Geometry: final body of the model. Coordinates: model frame, mm. A direction names the side the tool comes from. Coordinates: 2 decimals unless noted, no trailing zeros. Order: outer loops, then holes, each group sorted by start corner. A loop starts at its lowest first (then second) coordinate and runs counter-clockwise, first axis right, second up. Notation, with made-up numbers: M -14,-30 L 26,-30 A16 ccw 26,-20 Z; hole C 55.5,41 d10. An arc over 180 degrees is marked long. Use CSV: the item, a comma, the result in double quotes. Start each with the question number.
1. Section query C-C on z = 1.7. Return the cut outline in (x, y), and give its area (3 significant figures).
2. Set-up query: faces 1 (the flat face through (0, 0, 3)), 2 (the flat face through (13, -2.75, 2)). Return all of +Z, -Z, +X, -X, +Y, -Y with unobstructed straight access to the full face (end or side cutting, diameter ignored); none if empty.
3. First-contact query: P1, Ø1, axis at y = 5.5, z = 2.5, coming from the +X side; P2, Ø4.5, axis at x = -17.5, y = 0, coming from the -Z side. Flat tips, straight axial feed; report the tip coordinate or a pass-through.
4. Pull-direction query (Y, two-part tool) for faces 3 (the flat face through (21, 6, 1)), 4 (the flat face through (-21, -6, 1)), 5 (the cylindrical face through (20.25, 0.06, 1.52)), 6 (the cylindrical face through (4.75, -0.06, 1.52)); classes: pulls with the +Y half, pulls with the -Y half, needs draft (parallel to the pull), parting line crosses it, or undercut.
5. Section query A-A on x = 13.5. Return the cut outline in (y, z), and give its area (3 significant figures).
6. Section query B-B on y = 0. Return the cut outline in (x, z).
7. Section query D-D on x = -17.5. Return the cut outline in (y, z), and give its area (3 significant figures).
8. Material intervals for line 1 (Y direction, x = -17.5, z = 1.1); line 2 (X direction, y = 0.5, z = 0.9); line 3 (Y direction, x = 20, z = 0.25), sorted ascending.
from build123d import *

# Parameters (mm, degrees)
SKETCH1_W             = 45
SKETCH1_H             = 15
BOSS_EXTRUDE1_DEPTH   = 3
M4_TAPPED_HOLE1_D     = 3.3
M4_TAPPED_HOLE1_DEPTH = 10.1
M4_TAPPED_HOLE1_TIP   = 0.991420021
CUT_EXTRUDE1_DEPTH    = 3
CHAMFER1_SIZE         = 3
CHAMFER2_SIZE         = 0.5


with BuildPart() as part:
    # Sketch1 → Boss-Extrude1 (new body)
    with BuildSketch(Plane.XY):
        Rectangle(SKETCH1_W, SKETCH1_H)
    extrude(amount=BOSS_EXTRUDE1_DEPTH)

    # M4 Tapped Hole1
    with Locations(Plane.XY.offset(3)):
        with Locations((-17.5, 0)):
            Hole(M4_TAPPED_HOLE1_D / 2, depth=M4_TAPPED_HOLE1_DEPTH)
            with Locations((0, 0, -(M4_TAPPED_HOLE1_DEPTH + M4_TAPPED_HOLE1_TIP / 2))):  # 118° drill point
                Cone(0, M4_TAPPED_HOLE1_D / 2, M4_TAPPED_HOLE1_TIP, mode=Mode.SUBTRACT)

    # Sketch4 → Cut-Extrude1 (cut)
    with BuildSketch(Plane.XY.offset(3)):
        with BuildLine():
            Line((7.5, 2.75), (17.5, 2.75))
            ThreePointArc((17.5, 2.75), (20.25, 0), (17.5, -2.75))
            Line((17.5, -2.75), (7.5, -2.75))
            ThreePointArc((7.5, -2.75), (4.75, 0), (7.5, 2.75))
        make_face()
    extrude(amount=-CUT_EXTRUDE1_DEPTH, mode=Mode.SUBTRACT)

    # Chamfer1
    chamfer1_edges = [part.edges().sort_by_distance(p)[0] for p in [
        (22.5, -7.5, 1.5),
        (-22.5, -7.5, 1.5),
        (-22.5, 7.5, 1.5),
        (22.5, 7.5, 1.5),
    ]]
    chamfer(chamfer1_edges, length=CHAMFER1_SIZE)

    # Chamfer2
    chamfer2_edges = [part.edges().sort_by_distance(p)[0] for p in [
        (0, -7.5, 0),
        (0, 7.5, 0),
        (0, -7.5, 3),
        (0, 7.5, 3),
    ]]
    chamfer(chamfer2_edges, length=CHAMFER2_SIZE)


solid = part.part
Results list:
1,outline,"M -22.5,-4.5 L -19.5,-7.5 L 19.5,-7.5 L 22.5,-4.5 L 22.5,4.5 L 19.5,7.5 L -19.5,7.5 L -22.5,4.5 Z; hole C -17.5,0 d3.3; hole M 7.5,-2.75 L 17.5,-2.75 A2.75 ccw 17.5,2.75 L 7.5,2.75 A2.75 ccw Z"
1,area,"570 mm²"
2,face 1,"+Z, +X, -X, +Y, -Y"
2,face 2,"+Z, -Z"
3,P1,"stops at x = 22"
3,P2,"stops at z = 0"
4,face 3,"pulls with the +Y half"
4,face 4,"pulls with the -Y half"
4,face 5,"undercut"
4,face 6,"undercut"
5,outline,"M -7.5,0.5 L -7,0 L -2.75,0 L -2.75,3 L -7,3 L -7.5,2.5 Z; M 2.75,0 L 7,0 L 7.5,0.5 L 7.5,2.5 L 7,3 L 2.75,3 Z"
5,area,"28.0 mm²"
6,outline,"M -22.5,0 L -19.15,0 L -19.15,3 L -22.5,3 Z; M -15.85,0 L 4.75,0 L 4.75,3 L -15.85,3 Z; M 20.25,0 L 22.5,0 L 22.5,3 L 20.25,3 Z"
7,outline,"M -7.5,0.5 L -7,0 L -1.65,0 L -1.65,3 L -7,3 L -7.5,2.5 Z; M 1.65,0 L 7,0 L 7.5,0.5 L 7.5,2.5 L 7,3 L 1.65,3 Z"
7,area,"34.6 mm²"
8,line 1,"y = -7.5 to -1.65, 1.65 to 7.5"
8,line 2,"x = -22.5 to -19.07, -15.93 to 4.8, 20.2 to 22.5"
8,line 3,"y = -7 to -1.15, 1.15 to 7"
